Work out the finished part from the listing and answer in its coordinate system (mm). A direction names the side the tool comes from. Give positions to 0.01 mm unless a question says otherwise; leave off trailing zeros. Loops run counter-clockwise (first coordinate to the right, second up) from the corner with the lowest first, then second, coordinate; pieces in that order, holes last. Notation, with made-up numbers: M -33.5,15.5 L 0.5,15.5 A23 ccw 0.5,43.5 Z; hole C 77,19 d5. An arc over 180 degrees is marked long. Use a Markdown table: item, result.
```python
from build123d import *

# Parameters (mm, degrees)
CUT_EXTRUDE1_DEPTH = 2.5


with BuildPart() as part:
    # Sketch1 → Revolve1 (revolve)
    with BuildSketch(Plane(origin=(0, 0, 0), x_dir=(0, 0, -1), z_dir=(1, 0, 0))):
        Polygon((0, 185), (-10, 185), (-10, 145), (-20, 145), (-20, -145), (-10, -145), (-10, -185), (0, -185), align=None)
    revolve(axis=Axis((0, 189.929754582, 0), (0, -1, 0)))

    # Sketch2 → Cut-Extrude1 (cut)
    with BuildSketch(Plane(origin=(0, 0, -10), x_dir=(-1, 0, 0), z_dir=(0, 0, -1))):
        with BuildLine():
            Line((2.5, 175), (2.5, 155))
            ThreePointArc((2.5, 155), (0, 152.5), (-2.5, 155))
            Line((-2.5, 155), (-2.5, 175))
            ThreePointArc((-2.5, 175), (0, 177.5), (2.5, 175))
        make_face()
    cut_extrude1 = extrude(amount=-CUT_EXTRUDE1_DEPTH, mode=Mode.SUBTRACT)

    # Mirror1: Cut-Extrude1 across plane
    add(cut_extrude1.mirror(Plane.ZX), mode=Mode.SUBTRACT)


solid = part.part
```
(1) Given P1, Ø8, axis at y = -38.5, z = -2, coming from the +X side; P2, Ø10, axis at x = -7, y = 38.5, coming from the +Z side; P3, Ø4, axis at x = -11.5, y = -29, coming from the +Z side, each flat-ended and moving along its own axis, determine where each tip first touches the part or whether it passes through.
Entries:
| item | result |
|---|---|
| P1 | stops at x = 20 |
| P2 | stops at z = 19.9 |
| P3 | stops at z = 17.6 |
(2) A cutting plane is placed at B-B (y = -65.5). Write down the section's boundary in (x, z), and give its area (3 significant figures).
Entries:
| item | result |
|---|---|
| outline | C 0,0 d40 |
| area | 1,260 mm² |
(3) A cutting plane is placed at A-A (z = 0). Write down the section's boundary in (x, y), and give its area (3 significant figures).
Entries:
| item | result |
|---|---|
| outline | M -20,-145 L -10,-145 L -10,-185 L 10,-185 L 10,-145 L 20,-145 L 20,145 L 10,145 L 10,185 L -10,185 L -10,145 L -20,145 Z |
| area | 13,200 mm² |
(4) Which of the six approach directions +Z, -Z, +X, -X, +Y, -Y give full straight-line access (tool end or side, diameter ignored) to faces 1 (the cylindrical face through (3.83, -165.28, 9.237)), 2 (the flat face through (-9, 145, 5)), 3 (the flat face through (0, -185, 0))?
Entries:
| item | result |
|---|---|
| face 1 | -Y |
| face 2 | +Y |
| face 3 | +Z, -Z, +X, -X, -Y |
(5) A cutting plane is placed at C-C (z = 16). Write down the section's boundary in (x, y).
Entries:
| item | result |
|---|---|
| outline | M -12,-145 L 12,-145 L 12,145 L -12,145 Z |
(6) Consider probe 1 along Y at (x, z) = (-9, 17); probe 2 along X at (y, z) = (141.5, 1.5); probe 3 along Z at (x, y) = (4.5, 77). Determine where each line is inside the solid, lowest interval first. Write a range as [from, to].
Entries:
| item | result |
|---|---|
| probe 1 | y = [-145, 145] |
| probe 2 | x = [-19.94, 19.94] |
| probe 3 | z = [-19.49, 19.49] |
